Input: dimensioned drawing with shaded views. Units: mm. Origin: part minimum x, y, z. A direction names the side the tool comes from. Coordinates: 2 decimals unless noted, no trailing zeros. Loops run counter-clockwise (first coordinate to the right, second up) from the corner with the lowest first, then second, coordinate; pieces in that order, holes last.
(1) Mould query, pull axis Z, two halves, no side actions, for the marked faces 5, 6, 7 and 8. Classes: released by +Z, released by -Z, zero draft, split by the parting line, or undercut.
(2) Set-up query: the marked faces 1, 2, 3 and 4. Return all of +Z, -Z, +X, -X, +Y, -Y with unobstructed straight access to the full face (end or side cutting, diameter ignored); none if empty.
(3) Line query: L1, parallel to Y at x = 71, z = 19; L2, parallel to X at y = 35.5, z = 32.5; L3, parallel to X at y = 25.5, z = 15.5. Output: solid intervals per line, ascending.
(4) Contact query for flat-ended pins moving along their axis: P1, Ø2, axis at x = 52.5, z = 10, coming from the +Y side; P2, Ø11.5, axis at y = 16.5, z = 19, coming from the -X side; P3, Ø3.5, axis at x = 24.5, z = 19.5, coming from the -Y side. Output: stop coordinate, or through.
(5) Section B-B, the plane y = 45. Return loops of the section in (x, z) (1 decimal), then the cut area to 3 significant figures.
(6) Section C-C, the plane x = 12.5. Return loops of the section in (y, z), then the cut area to 3 significant figures.
(7) Section D-D, the plane y = 30. Return loops of the section in (x, z), then the cut area to 3 significant figures.
(8) Section A-A, the plane z = 19. Return loops of the section in (x, y), then the cut area to 3 significant figures.
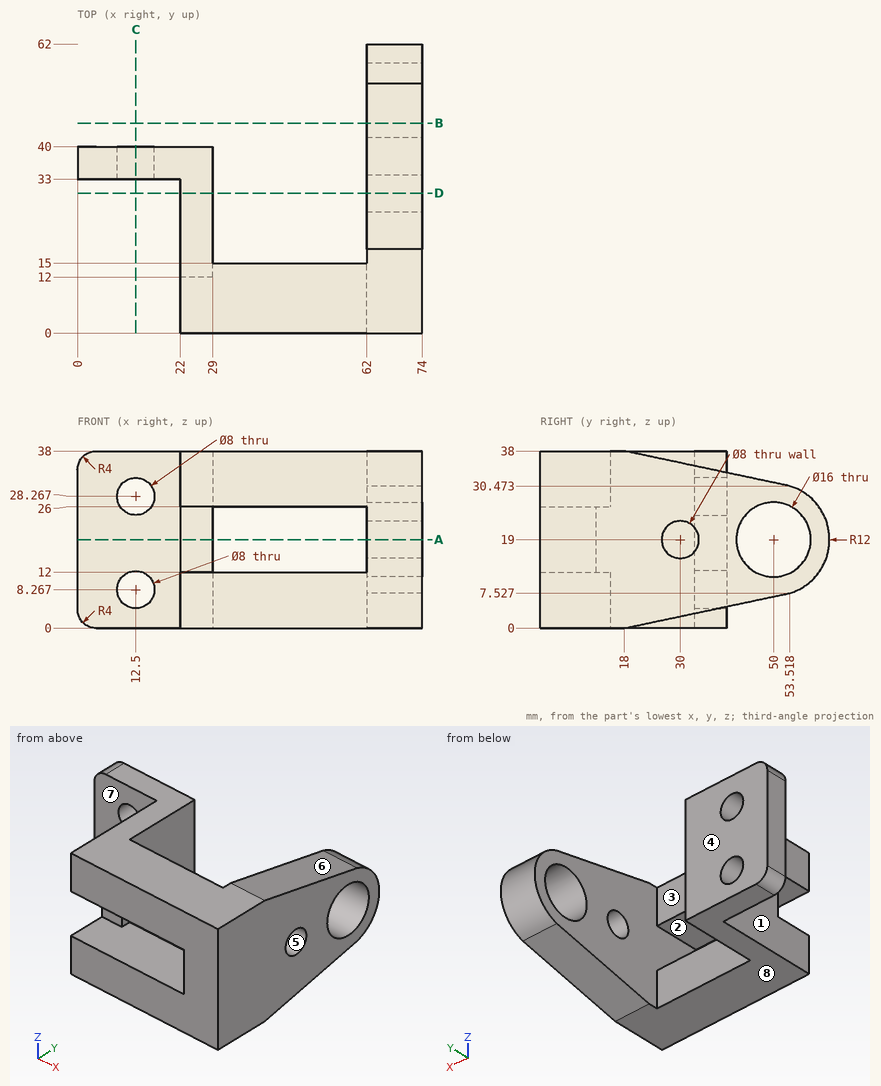
Report:
1. face 5: undercut
1. face 6: released by +Z
1. face 7: zero draft
1. face 8: released by -Z
2. face 1: +Z, -Z, -X, -Y
2. face 2: -Y
2. face 3: +Z, -Z, +Y
2. face 4: +Z, -Z, -X, +Y
3. L1: y = 0 to 26, 34 to 42, 58 to 62
3. L2: x = 0 to 29, 62 to 74
3. L3: x = 22 to 29, 62 to 74
4. P1: stops at y = 15
4. P2: stops at x = 22
4. P3: stops at y = 12
5. outline: (62, 5.7) - (74, 5.7) - (74, 12.8) - (62, 12.8) - close; (62, 25.2) - (74, 25.2) - (74, 32.3) - (62, 32.3) - close
5. area: 169 mm2
6. outline: (33, 0) - (40, 0) - (40, 4.27) - (33, 4.27) - close; (33, 12.27) - (40, 12.27) - (40, 24.27) - (33, 24.27) - close; (33, 32.27) - (40, 32.27) - (40, 38) - (33, 38) - close
6. area: 154 mm2
7. outline: (22, 0) - (29, 0) - (29, 38) - (22, 38) - close; (62, 2.54) - (74, 2.54) - (74, 15) - (62, 15) - close; (62, 23) - (74, 23) - (74, 35.46) - (62, 35.46) - close
7. area: 565 mm2
8. outline: (0, 33) - (22, 33) - (22, 12) - (29, 12) - (29, 40) - (0, 40) - close; (62, 0) - (74, 0) - (74, 26) - (62, 26) - close; (62, 34) - (74, 34) - (74, 42) - (62, 42) - close; (62, 58) - (74, 58) - (74, 62) - (62, 62) - close
8. area: 806 mm2
